from build123d import *

# Parameters (mm, degrees)
SKETCH1_R           = 5
BOSS_EXTRUDE1_DEPTH = 25
SKETCH2_R           = 6.5
BOSS_EXTRUDE2_DEPTH = 1
SKETCH3_R           = 4.25
BOSS_EXTRUDE3_DEPTH = 4.5
SKETCH4_R           = 3
BOSS_EXTRUDE4_DEPTH = 29
SKETCH6_W           = 1.7
SKETCH6_H           = 11.931395552
CUT_EXTRUDE1_DEPTH  = 3
BOSS_EXTRUDE5_START = 1
SKETCH7_R           = 6.5
BOSS_EXTRUDE5_DEPTH = 1


with BuildPart() as part:
    # Sketch1 → Boss-Extrude1 (new body)
    with BuildSketch(Plane.XY):
        Circle(SKETCH1_R)
    extrude(amount=BOSS_EXTRUDE1_DEPTH)

    # Sketch2 → Boss-Extrude2 (add)
    with BuildSketch(Plane.XY.offset(25)):
        Circle(SKETCH2_R)
    extrude(amount=BOSS_EXTRUDE2_DEPTH)

    # Sketch3 → Boss-Extrude3 (add)
    with BuildSketch(Plane.XY.offset(26)):
        with Locations((1.5, 0)):
            Circle(SKETCH3_R)
    extrude(amount=BOSS_EXTRUDE3_DEPTH)

    # Sketch4 → Boss-Extrude4 (add)
    with BuildSketch(Plane.XY.offset(30.5)):
        with Locations(Location((1.5, 0, 0), (0, 0, 180))):
            Circle(SKETCH4_R)
    extrude(amount=BOSS_EXTRUDE4_DEPTH)

    # Sketch6 → Cut-Extrude1 (cut)
    with BuildSketch(Plane(origin=(0, 0, 0), x_dir=(-1, 0, 0), z_dir=(0, 0, -1))):
        Rectangle(SKETCH6_W, SKETCH6_H)
    extrude(amount=-CUT_EXTRUDE1_DEPTH, mode=Mode.SUBTRACT)

    # Sketch7 → Boss-Extrude5 (add)
    with BuildSketch(Plane(origin=(0, 0, 25), x_dir=(-1, 0, 0), z_dir=(0, 0, -1)).offset(BOSS_EXTRUDE5_START)):
        Circle(SKETCH7_R)
    extrude(amount=-BOSS_EXTRUDE5_DEPTH)


solid = part.part
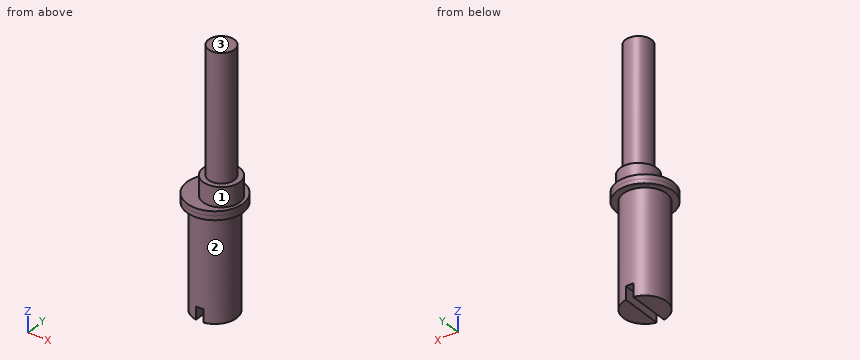
The model under review builds one solid part; all positions refer to its coordinate system, in mm. Face numbers are marked on the shaded views. A direction names the side the tool comes from. Round coordinates to 2 decimals unless told otherwise and drop trailing zeros. Loops run counter-clockwise (first coordinate to the right, second up) from the corner with the lowest first, then second, coordinate; pieces in that order, holes last. Notation, with made-up numbers: (23.5, -24.75) -> (58.5, -24.75) arc R5 ccw to (58.5, -20.75) -> close; hole circle Ø9 at (40, 51.25). An arc over 180 degrees is marked (long way). Return JSON: item names as keys, results as strings.
(1) Add section B-B on x = 0. Write out the cut boundary in (y, z).
Solved:
{"outline": "(-6.5, 24) -> (-5, 24) -> (-5, 3) -> (5, 3) -> (5, 24) -> (6.5, 24) -> (6.5, 26) -> (3.98, 26) -> (3.98, 30.5) -> (2.6, 30.5) -> (2.6, 59.5) -> (-2.6, 59.5) -> (-2.6, 30.5) -> (-3.98, 30.5) -> (-3.98, 26) -> (-6.5, 26) -> close"}
(2) Add section D-D on x = -2.25. Write out the cut boundary in (y, z).
Solved:
{"outline": "(-6.1, 24) -> (-4.47, 24) -> (-4.47, 0) -> (4.47, 0) -> (4.47, 24) -> (6.1, 24) -> (6.1, 26) -> (2, 26) -> (2, 30.5) -> (-2, 30.5) -> (-2, 26) -> (-6.1, 26) -> close"}
(3) For pin 1 (1.5 mm diameter, centred on y = 2.5, z = 36, fed in from -X); pin 2 (1 mm diameter, centred on x = 2, y = -4, fed in from +Z); pin 3 (1.5 mm diameter, centred on y = -1, z = 1.5, fed in from -X), all flat-tipped, find the tip position at first contact; note any pin that passes through.
Solved:
{"pin 1": "x = -0.94", "pin 2": "z = 30.5", "pin 3": "x = -4.99"}
(4) For the marked faces 1, 2 and 3, list the 3-axis set-ups (+Z, -Z, +X, -X, +Y, -Y) from which the entire face can be reached by the end or side of a thin tool; tool diameter is ignored.
Solved:
{"face 1": "+Z", "face 2": "-Z", "face 3": "+Z, +X, -X, +Y, -Y"}
(5) Add section C-C on z = 4. Write out the cut boundary in (x, y).
Solved:
{"outline": "circle Ø10 at (0, 0)"}
(6) Add section A-A on y = 0. Write out the cut boundary in (x, z), plus the area to 3 significant figures.
Solved:
{"outline": "(-6.5, 24) -> (-5, 24) -> (-5, 0) -> (-0.85, 0) -> (-0.85, 3) -> (0.85, 3) -> (0.85, 0) -> (5, 0) -> (5, 24) -> (6.5, 24) -> (6.5, 26) -> (5.75, 26) -> (5.75, 30.5) -> (4.5, 30.5) -> (4.5, 59.5) -> (-1.5, 59.5) -> (-1.5, 30.5) -> (-2.75, 30.5) -> (-2.75, 26) -> (-6.5, 26) -> close", "area": "473 mm2"}
(7) For line 1 (X direction, y = -4, z = 8.5); line 2 (Y direction, x = 1.75, z = 40); line 3 (Z direction, x = -0.5, y = -0.25), list the stretches that pass through material, from the lowest coordinate up.
Solved:
{"line 1": "-3 to 3", "line 2": "-2.99 to 2.99", "line 3": "3 to 59.5"}
